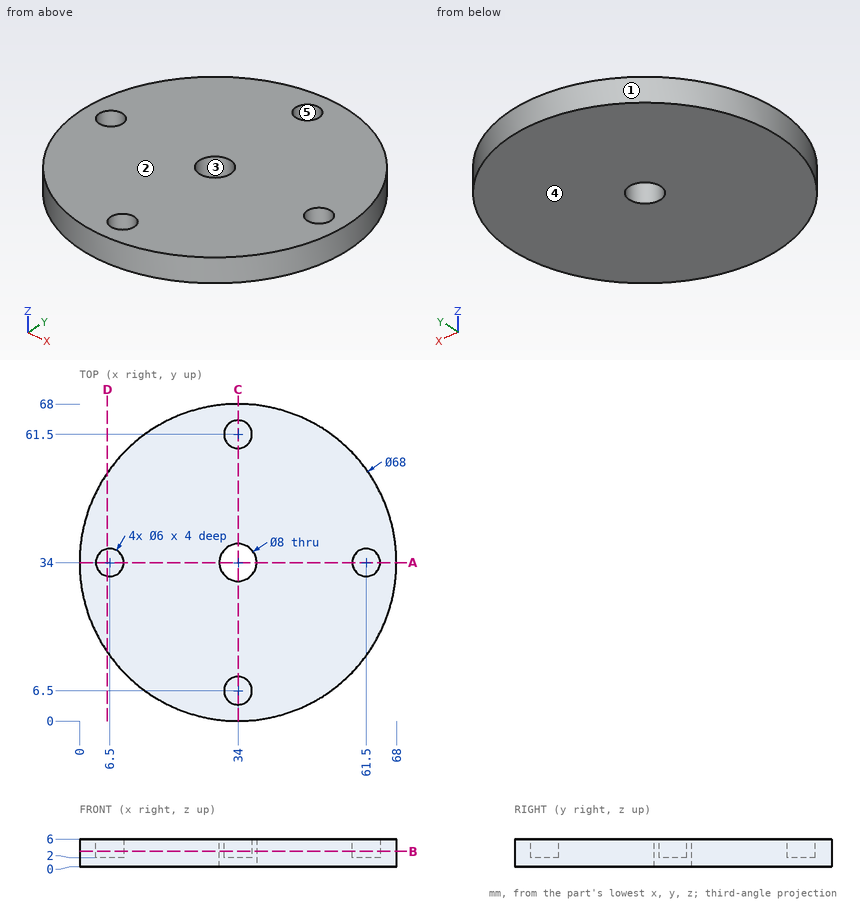
For this review, use the dimensioned drawing (mm, ordinates from the lowest corner) and the shaded views. A direction names the side the tool comes from. Round coordinates to 2 decimals unless told otherwise and drop trailing zeros. Write each loop counter-clockwise with the first axis right and the second up, starting at its lowest first coordinate (ties: lowest second). Pieces come first, ordered by that corner, then holes. Notation, with made-up numbers: (72, 33.5) - (105, 33.5) arc R23 ccw to (105, 55.5) - close; hole circle Ø6 at (48.5, -17). An arc over 180 degrees is marked (long way). Answer as CSV lines item,"result". Start each with the question number.
(1) Draft analysis for pull direction Y (two halves, no side actions). For the marked faces 1, 2 and 3, state which applies: pulls with the +Y half, pulls with the -Y half, needs draft (parallel to the pull), parting line crosses it, or undercut.
(2) We need section A-A on y = 34. State the section outline as (x, z) points.
(3) For the marked faces 4 and 5, list the 3-axis set-ups (+Z, -Z, +X, -X, +Y, -Y) from which the entire face can be reached by the end or side of a thin tool; tool diameter is ignored.
(4) We need section D-D on x = 6. State the section outline as (y, z) points, plus the area to 3 significant figures.
(5) For pin 1 Ø3.5 at (x, y) = (34, 6.5) entering from +Z; pin 2 Ø2 at (y, z) = (17.5, 5) entering from -X; pin 3 Ø7 at (x, y) = (34, 34) entering from -Z, all flat-tipped, find the tip position at first contact; note any pin that passes through.
(6) We need section B-B on z = 3.35. State the section outline as (x, y) points, plus the area to 3 significant figures.
(7) To check wall thickness, follow line 1 (Y direction, x = 34, z = 4.55); line 2 (Y direction, x = 6.5, z = 4.15); line 3 (X direction, y = 63.5, z = 3.95). State the ranges of each line that lie inside material, in increasing order.
Worked answers:
1,face 1,"parting line crosses it"
1,face 2,"needs draft"
1,face 3,"undercut"
2,outline,"(0, 0) - (30, 0) - (30, 6) - (9.5, 6) - (9.5, 2) - (3.5, 2) - (3.5, 6) - (0, 6) - close; (38, 0) - (68, 0) - (68, 6) - (64.5, 6) - (64.5, 2) - (58.5, 2) - (58.5, 6) - (38, 6) - close"
3,face 4,"-Z, +X, -X, +Y, -Y"
3,face 5,"+Z"
4,outline,"(14.71, 0) - (53.29, 0) - (53.29, 6) - (36.96, 6) - (36.96, 2) - (31.04, 2) - (31.04, 6) - (14.71, 6) - close"
4,area,"208 mm²"
5,pin 1,"z = 2"
5,pin 2,"x = 3.74"
5,pin 3,"through"
6,outline,"circle Ø68 at (34, 34); hole circle Ø6 at (6.5, 34); hole circle Ø8 at (34, 34); hole circle Ø6 at (34, 6.5); hole circle Ø6 at (34, 61.5); hole circle Ø6 at (61.5, 34)"
6,area,"3,470 mm²"
7,line 1,"0 to 3.5, 9.5 to 30, 38 to 58.5, 64.5 to 68"
7,line 2,"14.01 to 31, 37 to 53.99"
7,line 3,"17.1 to 31.76, 36.24 to 50.9"
